Work out the finished part from the listing and answer in its coordinate system (mm). Coordinates: 2 decimals unless noted, no trailing zeros. Loops run counter-clockwise (first coordinate to the right, second up) from the corner with the lowest first, then second, coordinate; pieces in that order, holes last. Notation, with made-up numbers: (0, 38.5) -> (22, 38.5) arc R27 cw to (22, 56.5) -> close; hole circle Ø4 at (46, 15). An arc over 180 degrees is marked (long way). Use a Markdown table: item, result. Add a question column.
```python
from build123d import *

# Parameters (mm, degrees)
SKETCH1_R           = 8
SKETCH1_R_2         = 6.25
BOSS_EXTRUDE1_DEPTH = 2
CHAMFER1_SIZE       = 0.2


with BuildPart() as part:
    # Sketch1 → Boss-Extrude1 (new, symmetric)
    with BuildSketch(Plane.XY):
        Circle(SKETCH1_R)
        Circle(SKETCH1_R_2, mode=Mode.SUBTRACT)
    extrude(amount=BOSS_EXTRUDE1_DEPTH, both=True)

    # Chamfer1
    chamfer1_edges = [part.edges().sort_by_distance(p)[0] for p in [
        (-8, 0, -2),
        (-8, 0, 2),
        (-6.25, 0, -2),
        (-6.25, 0, 2),
    ]]
    chamfer(chamfer1_edges, length=CHAMFER1_SIZE)


solid = part.part
```
Item 1: Find the intervals of material crossed by probe 1 along Y at (x, z) = (0, -0.3); probe 2 along Y at (x, z) = (5.75, 1.1); probe 3 along X at (y, z) = (1.5, -1.4), in increasing order.
Item 2: Section C-C (z = 0.05) is taken. Determine the outline of the cut face in (x, y).
Item 3: Given pin 1 (6 mm diameter, centred on x = 0, y = -0.5, fed in from +Z); pin 2 (2 mm diameter, centred on y = 4.5, z = 0.5, fed in from +X); pin 3 (6 mm diameter, centred on x = 5, y = 1.5, fed in from +Z), each flat-ended and moving along its own axis, determine where each tip first touches the part or whether it passes through.
Item 4: For a pull along Y with two mould halves and no side action, classify faces 1 (the face through (-1.73, -7.81, 0.03)), 2 (the face through (-3, 6, -2)), 3 (the face through (5.96, 1.88, -0.03)) as +Y half, -Y half, draft (parallel to the pull), parting line (faces both ways), or undercut.
Item 5: Section A-A (y = 0) is taken. Determine the outline of the cut face in (x, z).
Output:
| question | item | result |
|---|---|---|
| 1 | probe 1 | y = -8 to -6.25, 6.25 to 8 |
| 1 | probe 2 | y = -5.56 to -2.45, 2.45 to 5.56 |
| 1 | probe 3 | x = -7.86 to -6.07, 6.07 to 7.86 |
| 2 | outline | circle Ø16 at (0, 0); hole circle Ø12.5 at (0, 0) |
| 3 | pin 1 | passes through |
| 3 | pin 2 | stops at x = 7.19 |
| 3 | pin 3 | stops at z = 2 |
| 4 | face 1 | parting line |
| 4 | face 2 | draft |
| 4 | face 3 | undercut |
| 5 | outline | (-8, -1.8) -> (-7.8, -2) -> (-6.45, -2) -> (-6.25, -1.8) -> (-6.25, 1.8) -> (-6.45, 2) -> (-7.8, 2) -> (-8, 1.8) -> close; (6.25, -1.8) -> (6.45, -2) -> (7.8, -2) -> (8, -1.8) -> (8, 1.8) -> (7.8, 2) -> (6.45, 2) -> (6.25, 1.8) -> close |
